Verification items for the finished model (mm, model axes). A direction names the side the tool comes from. Coordinates: 2 decimals unless noted, no trailing zeros. Loops run counter-clockwise (first coordinate to the right, second up) from the corner with the lowest first, then second, coordinate; pieces in that order, holes last. Notation, with made-up numbers: (59, 30.5) - (114, 30.5) arc R17 ccw to (114, 49.5) - close; hole circle Ø10 at (63, 59). An arc over 180 degrees is marked (long way). One line per item, written item: value. Start each with the question number.
(1) Section check D-D (y = 18). Record the boundary of the cut face in (x, z), plus the area to 3 significant figures.
(2) Gauge pin test, flat ends, axial feed: P1, Ø1, axis at y = -10, z = -13.5, coming from the -X side; P2, Ø2, axis at x = 357.5, y = -6.5, coming from the +Z side; P3, Ø23.5, axis at y = -2, z = 8.5, coming from the -X side; P4, Ø2, axis at y = 1, z = -10, coming from the -X side. Record the tip position at first contact, or that the pin passes through.
(3) Thickness scan on probe 1 along Z at (x, y) = (22, 1); probe 2 along Y at (x, z) = (210, -1); probe 3 along X at (y, z) = (0.5, -9.5). Record the ranges inside material, lowest first. Write a range as [from, to].
(4) Section check C-C (x = 149.5). Record the boundary of the cut face in (y, z), plus the area to 3 significant figures.
(5) Section check A-A (z = 0). Record the boundary of the cut face in (x, y).
(6) Set-up check for faces 1 (the face through (435.14, -6.324, -4.032)), 2 (the face through (21, 0, 10)), 3 (the face through (225.3, -23.3, 3.06)): record each of +Z, -Z, +X, -X, +Y, -Y from which the full face is reachable in a straight line by a thin tool's end or side.
```python
from build123d import *


with BuildPart() as part:
    # Sketch1 → Revolve1 (revolve)
    with BuildSketch(Plane.XY, mode=Mode.PRIVATE) as revolve1_sk:
        Polygon((0, 0), (0, 7.5), (20, 7.5), (20, 10), (22.5, 10), (22.5, 23.5), (422.5, 23.5), (422.5, 10), (425, 10), (425, 7.5), (445, 7.5), (445, 0), align=None)
    revolve(revolve1_sk.sketch.rotate(Axis((0, 0, 0), (-1, 0, 0)), 90), axis=Axis((0, 0, 0), (-1, 0, 0)))


solid = part.part
```
Responses:
1. outline: (22.5, -15.11) - (422.5, -15.11) - (422.5, 15.11) - (22.5, 15.11) - close
1. area: 12,100 mm²
2. P1: stops at x = 22.5
2. P2: stops at z = 22.85
2. P3: stops at x = 0
2. P4: stops at x = 20
3. probe 1: z = [-9.95, 9.95]
3. probe 2: y = [-23.48, 23.48]
3. probe 3: x = [20, 425]
4. outline: circle Ø47 at (0, 0)
4. area: 1,730 mm²
5. outline: (0, -7.5) - (20, -7.5) - (20, -10) - (22.5, -10) - (22.5, -23.5) - (422.5, -23.5) - (422.5, -10) - (425, -10) - (425, -7.5) - (445, -7.5) - (445, 7.5) - (425, 7.5) - (425, 10) - (422.5, 10) - (422.5, 23.5) - (22.5, 23.5) - (22.5, 10) - (20, 10) - (20, 7.5) - (0, 7.5) - close
6. face 1: +X
6. face 2: -X
6. face 3: +X, -X
